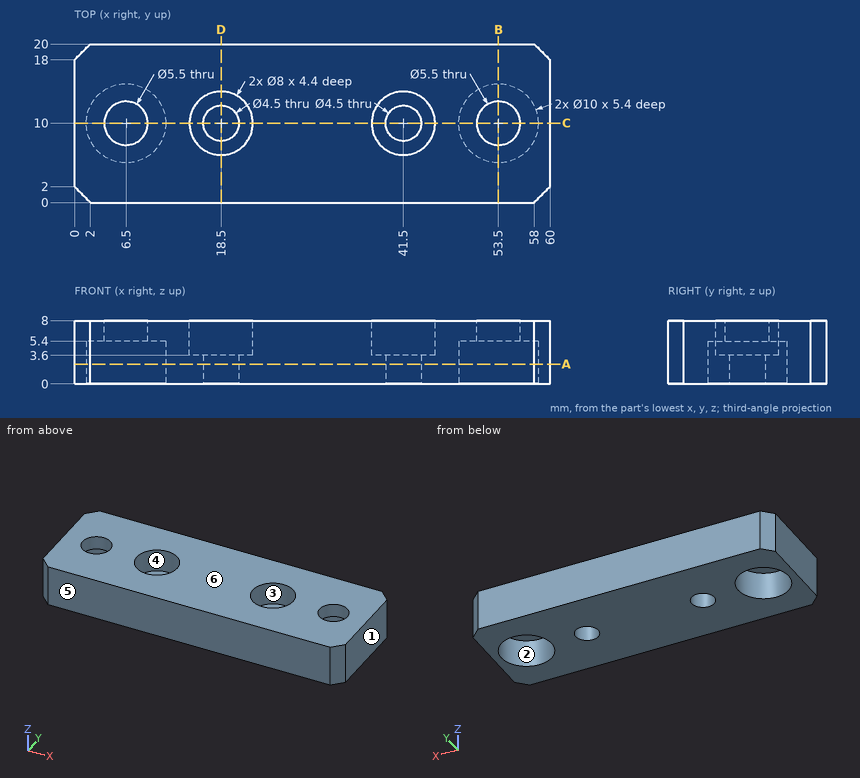
Design review of the part shown in the three views and the two pictorial views. Dimensions are in mm from the part's minimum x, y and z. A direction names the side the tool comes from. Give positions to 0.01 mm unless a question says otherwise; leave off trailing zeros. Loops run counter-clockwise (first coordinate to the right, second up) from the corner with the lowest first, then second, coordinate; pieces in that order, holes last. Notation, with made-up numbers: M 13.5,55.25 L 69.5,55.25 A16 ccw 69.5,63.25 Z; hole C 46,21.25 d11. An arc over 180 degrees is marked long. Put each result on its own line as item: value. Start each with the question number.
(1) Add section A-A, the plane z = 2.5. Write out the cut boundary in (x, y), then the cut area to 3 significant figures.
(2) Wall thickness on L1, parallel to Y at x = 53.5, z = 7.15; L2, parallel to X at y = 5.75, z = 4.5; L3, parallel to Y at x = 41.5, z = 1.5: over which ranges is each line inside the solid? List them lowest first.
(3) For pin 1 (6.5 mm diameter, centred on x = 41.5, y = 10, fed in from +Z); pin 2 (5 mm diameter, centred on x = 53.5, y = 10, fed in from +Z); pin 3 (8 mm diameter, centred on x = 53, y = 10, fed in from -Z), all flat-tipped, find the tip position at first contact; note any pin that passes through.
(4) Add section C-C, the plane y = 10. Give the number of separate pieces and of enclosed holes in the cut face, then the cut area to 3 significant figures.
(5) Add section D-D, the plane x = 18.5. Write out the cut boundary in (y, z), then the cut area to 3 significant figures.
(6) Add section B-B, the plane x = 53.5. Write out the cut boundary in (y, z).
(7) The part is to be moulded in two halves that separate along Y. For the marked faces 4, 5 and 6, say which applies: +Y half, -Y half, draft (parallel to the pull), parting line (faces both ways), or undercut.
(8) Machinability: for the marked faces 1, 2 and 3, which of the approach directions +Z, -Z, +X, -X, +Y, -Y give a long, thin tool a straight path to every point of the face, cutting with its end or side? Answer none if there is none.
Result:
1. outline: M 0,2 L 2,0 L 58,0 L 60,2 L 60,18 L 58,20 L 2,20 L 0,18 Z; hole C 6.5,10 d10; hole C 18.5,10 d4.5; hole C 41.5,10 d4.5; hole C 53.5,10 d10
1. area: 1,000 mm^2
2. L1: y = 0 to 7.25, 12.75 to 20
2. L2: x = 0 to 3.87, 9.13 to 50.87, 56.13 to 60
2. L3: y = 0 to 7.75, 12.25 to 20
3. pin 1: stops at z = 3.6
3. pin 2: passes through
3. pin 3: stops at z = 5.4
4. separate pieces: 5
4. enclosed holes: 0
4. area: 241 mm^2
5. outline: M 0,0 L 7.75,0 L 7.75,3.6 L 6,3.6 L 6,8 L 0,8 Z; M 12.25,0 L 20,0 L 20,8 L 14,8 L 14,3.6 L 12.25,3.6 Z
5. area: 109 mm^2
6. outline: M 0,0 L 5,0 L 5,5.4 L 7.25,5.4 L 7.25,8 L 0,8 Z; M 12.75,5.4 L 15,5.4 L 15,0 L 20,0 L 20,8 L 12.75,8 Z
7. face 4: undercut
7. face 5: -Y half
7. face 6: draft
8. face 1: +Z, -Z, +X, +Y, -Y
8. face 2: -Z
8. face 3: +Z
